Could you check a few things on this model? Use its own coordinates, in mm. Face numbers are marked on the shaded views. A direction names the side the tool comes from. Round coordinates to 2 decimals unless told otherwise and drop trailing zeros. Loops run counter-clockwise (first coordinate to the right, second up) from the corner with the lowest first, then second, coordinate; pieces in that order, holes last. Notation, with made-up numbers: M -13.5,-17.75 L 31.5,-17.75 A21 ccw 31.5,16.25 Z; hole C 8,40 d2. An arc over 180 degrees is marked long. One line per item, written item: value. Start each with the question number.
Q1. Which directions (+Z, -Z, +X, -X, +Y, -Y) give clear straight access to the entire face, cutting with the end or side of a thin tool? Please do the marked faces 5 and 6.
Q2. Please list where these lines run through material, in increasing order: line 1 along Y through (x, z) = (4.55, 0); line 2 along X through (y, z) = (-7, 2.75); line 3 along Y through (x, z) = (0.35, 7.5).
Q3. I'm going to push flat-ended pins straight in: pin 1 Ø1 at (x, y) = (1.5, 1.5) entering from -Z; pin 2 Ø2 at (x, y) = (4, -3.5) entering from +Z; pin 3 Ø1.5 at (y, z) = (2.5, 5) entering from +X. Where does each tip first touch, or does it pass through?
Q4. Imagine slicing it at C-C (x = 1.4). Please give me the cut outline in (y, z), then the cut area to 3 significant figures.
Q5. Thinking about a two-plate mould opening in Y: for the marked faces 1, 2, 3 and 4, which applies, released by +Y, released by -Y, zero draft, split by the parting line, or undercut?
from build123d import *


with BuildPart() as part:
    # 草图1 → 旋转1 (revolve)
    with BuildSketch(Plane.XY, mode=Mode.PRIVATE) as revolve_1_sk:
        with BuildLine():
            Line((0, 9.2), (0, 8.25))
            Line((0, 8.25), (0.3984, 8.25))
            Line((0.3984, 8.25), (0.3984, 4.25))
            Line((0.3984, 4.25), (0, 4.25))
            Line((0, 4.25), (0, 2.8))
            ThreePointArc((0, 2.8), (0.087867966, 2.587867966), (0.3, 2.5))
            Line((0.3, 2.5), (5.7, 2.5))
            ThreePointArc((5.7, 2.5), (5.912132034, 2.587867966), (6, 2.8))
            Line((6, 2.8), (6, 4.25))
            Line((6, 4.25), (5.6016, 4.25))
            Line((5.6016, 4.25), (5.6016, 8.25))
            Line((5.6016, 8.25), (6, 8.25))
            Line((6, 8.25), (6, 9.2))
            ThreePointArc((6, 9.2), (5.912132034, 9.412132034), (5.7, 9.5))
            Line((5.7, 9.5), (0.3, 9.5))
            ThreePointArc((0.3, 9.5), (0.087867966, 9.412132034), (0, 9.2))
        make_face()
    revolve(revolve_1_sk.sketch.rotate(Axis((5.7, 0, 0), (-1, 0, 0)), 270), axis=Axis((5.7, 0, 0), (-1, 0, 0)))


solid = part.part
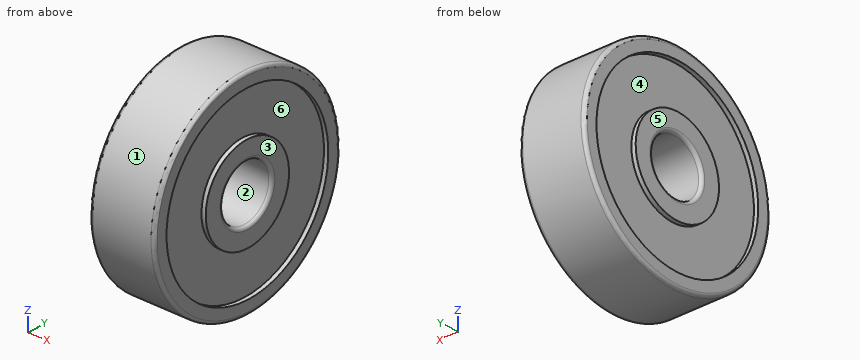
Report:
1. face 5: +Z, -Z, -X, +Y, -Y
1. face 6: +X
2. line 1: y = -9.5 to -2.5, 2.5 to 9.5
2. line 2: x = 0.4 to 5.6
2. line 3: y = -5.83 to -3.44, 3.44 to 5.83
3. pin 1: stops at z = -9.45
3. pin 2: stops at z = 9.17
3. pin 3: stops at x = 5.6
4. outline: C 0,0 d19; hole C 0,0 d5
4. area: 264 mm²
5. face 1: split by the parting line
5. face 2: undercut
5. face 3: zero draft
5. face 4: undercut
